```python
from build123d import *

# Parameters (mm, degrees)
SKETCH_1_R      = 5
SKETCH_1_R_2    = 3.2
EXTRUDE_1_DEPTH = 6
SKETCH_2_R      = 7
SKETCH_2_R_2    = 3.2
EXTRUDE_2_DEPTH = 5


with BuildPart() as part:
    # 草图1 → 凸台-拉伸1 (new, symmetric)
    with BuildSketch(Plane.XY):
        Circle(SKETCH_1_R)
        Circle(SKETCH_1_R_2, mode=Mode.SUBTRACT)
    extrude(amount=EXTRUDE_1_DEPTH, both=True)

    # 草图2 → 凸台-拉伸2 (add)
    with BuildSketch(Plane.XY):
        Circle(SKETCH_2_R)
        Circle(SKETCH_2_R_2, mode=Mode.SUBTRACT)
    extrude(amount=EXTRUDE_2_DEPTH)


solid = part.part
```
Here's how the part is built. I have some questions about the finished solid (model axes, mm). A direction names the side the tool comes from. Give positions to 0.01 mm unless a question says otherwise; leave off trailing zeros. Write each loop counter-clockwise with the first axis right and the second up, starting at its lowest first coordinate (ties: lowest second). Pieces come first, ordered by that corner, then holes. Notation, with made-up numbers: (-21.5, -15) -> (26.5, -15) arc R36 cw to (26.5, 22) -> close; hole circle Ø10 at (52.5, -20). An arc over 180 degrees is marked (long way). Write each question's results on one line, items separated by ' | '.
Item 1: On a 3-axis mill with a long thin cutter (end or side, diameter ignored), from which of +Z, -Z, +X, -X, +Y, -Y can I reach the whole of each face in a straight line? I mean faces 4 (the face through (1, -3.3, 6)), 5 (the face through (-1.08, -4.88, 5.51)), 6 (the face through (-2, 5, 0)). Say none if no direction works.
Output:
face 4: +Z, +X, -X, +Y, -Y | face 5: +Z | face 6: -Z
Item 2: We'd pull the mould along X, two halves only. Please class faces 1 (the face through (6.466, -2.681, 2.465)), 2 (the face through (1, -3.3, -6)), 3 (the face through (-2.539, -1.947, -0.084)): pulls with the +X half, pulls with the -X half, needs draft (parallel to the pull), parting line crosses it, or undercut.
Output:
face 1: parting line crosses it | face 2: needs draft | face 3: undercut
Item 3: If I drill on L1, parallel to Y at x = 0, z = -1; L2, parallel to Z at x = 3.5, y = 5; L3, parallel to X at y = -1.25, z = -0.5, over which ranges is the centre line in solid material (lowest first)?
Output:
L1: y = -5 to -3.2, 3.2 to 5 | L2: z = 0 to 5 | L3: x = -4.84 to -2.95, 2.95 to 4.84
Item 4: Suppose I cut it at C-C on z = 1.5. Write out the boundary of the cut face in (x, y), plus the area to 3 significant figures.
Output:
outline: circle Ø14 at (0, 0); hole circle Ø6.4 at (0, 0) | area: 122 mm^2
Item 5: Suppose I cut it at A-A on y = 0. Write out the boundary of the cut face in (x, z).
Output:
outline: (-7, 0) -> (-5, 0) -> (-5, -6) -> (-3.2, -6) -> (-3.2, 6) -> (-5, 6) -> (-5, 5) -> (-7, 5) -> close; (3.2, -6) -> (5, -6) -> (5, 0) -> (7, 0) -> (7, 5) -> (5, 5) -> (5, 6) -> (3.2, 6) -> close
Item 6: For pin 1 Ø3 at (x, y) = (0.5, 0) entering from -Z; pin 2 Ø1 at (y, z) = (1.5, -4) entering from -X; pin 3 Ø2 at (x, z) = (-3, 2.5) entering from -Y, each with a flat end and sliding along its axis, tell me the tip position at first contact or that it passes through.
Output:
pin 1: passes through | pin 2: stops at x = -4.9 | pin 3: stops at y = -6.71
Item 7: Suppose I cut it at D-D on x = -4. Write out the boundary of the cut face in (y, z), plus the area to 3 significant figures.
Output:
outline: (-5.74, 0) -> (-3, 0) -> (-3, -6) -> (3, -6) -> (3, 0) -> (5.74, 0) -> (5.74, 5) -> (3, 5) -> (3, 6) -> (-3, 6) -> (-3, 5) -> (-5.74, 5) -> close | area: 99.4 mm^2
